from build123d import *
from OCP.BRepFilletAPI import BRepFilletAPI_MakeChamfer

# Parameters (mm, degrees)
SKETCH_1_R          = 8
EXTRUDE_1_DEPTH     = 10
CUT_EXTRUDE_1_DEPTH = 5
SKETCH_3_R          = 5
EXTRUDE_2_DEPTH     = 10
CHAMFER_1_SIZE      = 1.25
FILLET_1_R          = 1.230769231
CHAMFER_2_SIZE      = 2.305475504
CHAMFER_2_SIZE2     = 3.993200709
FILLET_2_R          = 0.1


with BuildPart() as part:
    # 草图1 → 凸台-拉伸1 (new body)
    with BuildSketch(Plane.XY):
        Circle(SKETCH_1_R)
    extrude(amount=EXTRUDE_1_DEPTH)

    # 草图2 → 切除-拉伸1 (cut)
    with BuildSketch(Plane.XY.offset(10)):
        Polygon((4, 2.309401077), (0, 4.618802154), (-4, 2.309401077), (-4, -2.309401077), (0, -4.618802154), (4, -2.309401077), align=None)
    extrude(amount=-CUT_EXTRUDE_1_DEPTH, mode=Mode.SUBTRACT)

    # 草图3 → 凸台-拉伸2 (add)
    with BuildSketch(Plane(origin=(0, 0, 0), x_dir=(-1, 0, 0), z_dir=(0, 0, -1))):
        with Locations(Location((0, 0, 0), (0, 0, 180))):
            Circle(SKETCH_3_R)
    extrude(amount=EXTRUDE_2_DEPTH)

    # 倒角1
    chamfer_1_edges = [part.edges().sort_by_distance(p)[0] for p in [
        (-5, 0, -10),
    ]]
    chamfer(chamfer_1_edges, length=CHAMFER_1_SIZE)

    # 圆角1
    fillet_1_edges = [part.edges().sort_by_distance(p)[0] for p in [
        (-8, 0, 10),
    ]]
    fillet(fillet_1_edges, radius=FILLET_1_R)

    # 倒角2: one chamfer whose edges measure the first distance from different faces: ONE call of the kernel's chamfer builder (chamfer() names one face for all edges)
    chamfer_2_edges_1 = [part.edges().sort_by_distance(p)[0] for p in [
        (2, 3.464101615, 5),
    ]]
    chamfer_2_side_1 = [part.faces().sort_by_distance(p)[0] for p in [
        (2, 3.464101615, 7.5),
    ]]
    chamfer_2_edges_2 = [part.edges().sort_by_distance(p)[0] for p in [
        (4, 0, 5),
    ]]
    chamfer_2_side_2 = [part.faces().sort_by_distance(p)[0] for p in [
        (4, 0, 7.5),
    ]]
    chamfer_2_edges_3 = [part.edges().sort_by_distance(p)[0] for p in [
        (2, -3.464101615, 5),
    ]]
    chamfer_2_side_3 = [part.faces().sort_by_distance(p)[0] for p in [
        (2, -3.464101615, 7.5),
    ]]
    chamfer_2_edges_4 = [part.edges().sort_by_distance(p)[0] for p in [
        (-2, -3.464101615, 5),
    ]]
    chamfer_2_side_4 = [part.faces().sort_by_distance(p)[0] for p in [
        (-2, -3.464101615, 7.5),
    ]]
    chamfer_2_edges_5 = [part.edges().sort_by_distance(p)[0] for p in [
        (-4, 0, 5),
    ]]
    chamfer_2_side_5 = [part.faces().sort_by_distance(p)[0] for p in [
        (-4, 0, 7.5),
    ]]
    chamfer_2_edges_6 = [part.edges().sort_by_distance(p)[0] for p in [
        (-2, 3.464101615, 5),
    ]]
    chamfer_2_side_6 = [part.faces().sort_by_distance(p)[0] for p in [
        (-2, 3.464101615, 7.5),
    ]]
    chamfer_2 = BRepFilletAPI_MakeChamfer(part.part.solid().wrapped)
    for e in chamfer_2_edges_1:
        chamfer_2.Add(CHAMFER_2_SIZE, CHAMFER_2_SIZE2, e.wrapped, chamfer_2_side_1[0].wrapped)  # the first distance lies on this face
    for e in chamfer_2_edges_2:
        chamfer_2.Add(CHAMFER_2_SIZE, CHAMFER_2_SIZE2, e.wrapped, chamfer_2_side_2[0].wrapped)  # the first distance lies on this face
    for e in chamfer_2_edges_3:
        chamfer_2.Add(CHAMFER_2_SIZE, CHAMFER_2_SIZE2, e.wrapped, chamfer_2_side_3[0].wrapped)  # the first distance lies on this face
    for e in chamfer_2_edges_4:
        chamfer_2.Add(CHAMFER_2_SIZE, CHAMFER_2_SIZE2, e.wrapped, chamfer_2_side_4[0].wrapped)  # the first distance lies on this face
    for e in chamfer_2_edges_5:
        chamfer_2.Add(CHAMFER_2_SIZE, CHAMFER_2_SIZE2, e.wrapped, chamfer_2_side_5[0].wrapped)  # the first distance lies on this face
    for e in chamfer_2_edges_6:
        chamfer_2.Add(CHAMFER_2_SIZE, CHAMFER_2_SIZE2, e.wrapped, chamfer_2_side_6[0].wrapped)  # the first distance lies on this face
    add(Compound.cast(chamfer_2.Shape()), mode=Mode.REPLACE)

    # 圆角2
    fillet_2_edges = [part.edges().sort_by_distance(p)[0] for p in [
        (-5, 0, 0),
    ]]
    fillet(fillet_2_edges, radius=FILLET_2_R)


solid = part.part
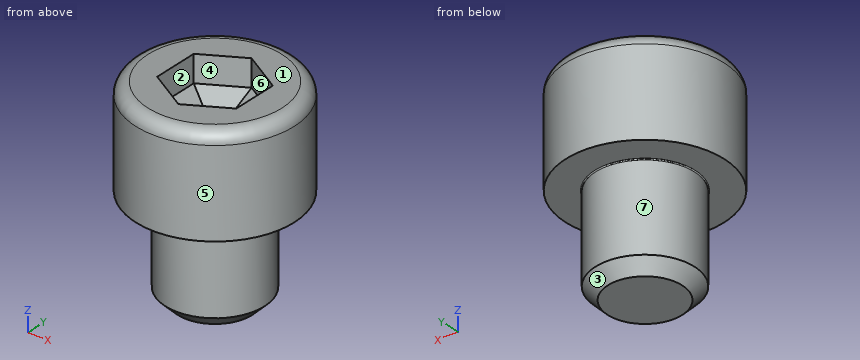
CAD build for the part. Positions are in the model's coordinates, mm. Face numbers are marked on the shaded views. A direction names the side the tool comes from. Coordinates: 2 decimals unless noted, no trailing zeros. Order: outer loops, then holes, each group sorted by start corner. A loop starts at its lowest first (then second) coordinate and runs counter-clockwise, first axis right, second up.
Item 1: Drill centre lines: L1, parallel to Z at x = -5, y = -4.5; L2, parallel to X at y = -0.25, z = 7; L3, parallel to Y at x = 2.75, z = 9. Where is each one in solid material? Low to high.
Check sheet entries:
L1: z = 0 to 10
L2: x = -8 to -3.47, 3.47 to 8
L3: y = -7.49 to -3.03, 3.03 to 7.49
Item 2: Band-saw the part on A-A on z = 4.25. List the corners of the cut face in (x, y).
Check sheet entries:
outline: circle Ø16 at (0, 0)
Item 3: Two-plate mould, pull along Y, no slides. Class the marked faces 1, 2, 3 and 4: +Y half, -Y half, draft (parallel to the pull), parting line (faces both ways), or undercut.
Check sheet entries:
face 1: draft
face 2: undercut
face 3: parting line
face 4: undercut
Item 4: Band-saw the part on B-B on z = -4.5. List the corners of the cut face in (x, y).
Check sheet entries:
outline: circle Ø10 at (0, 0)
Item 5: Pin check, flat tips, straight feed: pin 1 Ø1.5 at (y, z) = (1.5, -7) entering from +X; pin 2 Ø8 at (y, z) = (-6, 4) entering from -X; pin 3 Ø6 at (x, z) = (-5, -7.5) entering from +Y. Stop position of each tip, or through.
Check sheet entries:
pin 1: stops at x = 4.94
pin 2: stops at x = -7.75
pin 3: stops at y = 4.58
Item 6: 3-axis set-ups, long thin cutter, end or side, ignore diameter. For the marked faces 5, 6 and 7: which of +Z, -Z, +X, -X, +Y, -Y reach the whole face in a straight line?
Check sheet entries:
face 5: +Z, -Z
face 6: +Z
face 7: -Z
